Check sheet for the modelled part. Datum: model origin and axes. Units: mm. A direction names the side the tool comes from. Round coordinates to 2 decimals unless told otherwise and drop trailing zeros. Order: outer loops, then holes, each group sorted by start corner. A loop starts at its lowest first (then second) coordinate and runs counter-clockwise, first axis right, second up. Notation, with made-up numbers: (-24.5, -32.5) -> (-13.5, -32.5) arc R26 cw to (-13.5, -18.5) -> close; hole circle Ø11 at (36, -16). An arc over 180 degrees is marked (long way). Answer in a Markdown table with one row per item.
from build123d import *

# Parameters (mm, degrees)
SKETCH2_R           = 0.4
BOSS_EXTRUDE1_DEPTH = 0.5
SKETCH4_R           = 1
SKETCH4_R_2         = 0.5
CUT_EXTRUDE3_DEPTH  = 6


with BuildPart() as part:
    # Sketch1 → Revolve1 (revolve)
    with BuildSketch(Plane.XY, mode=Mode.PRIVATE) as revolve1_sk:
        Polygon((0, 0), (0, 1.5), (3, 1.5), (3, 1), (13, 1), (13, 0), align=None)
    revolve(revolve1_sk.sketch.rotate(Axis((0.124352332, 0, 0), (1, 0, 0)), 90), axis=Axis((0.124352332, 0, 0), (1, 0, 0)))

    # Sketch2 → Boss-Extrude1 (add, symmetric)
    with BuildSketch(Plane.XY):
        with BuildLine():
            Line((0, 0.75), (0, -0.75))
            Line((0, -0.75), (-3, -0.75))
            ThreePointArc((-3, -0.75), (-3.75, 0), (-3, 0.75))
            Line((-3, 0.75), (0, 0.75))
        make_face()
        with Locations((-3, 0)):
            Circle(SKETCH2_R, mode=Mode.SUBTRACT)
    extrude(amount=BOSS_EXTRUDE1_DEPTH, both=True)

    # Sketch4 → Cut-Extrude3 (cut)
    with BuildSketch(Plane(origin=(13, 0, 0), x_dir=(0, 0, -1), z_dir=(1, 0, 0))):
        with Locations(Location((0, 0, 0), (0, 0, 180))):
            Circle(SKETCH4_R)
        Circle(SKETCH4_R_2, mode=Mode.SUBTRACT)
    extrude(amount=-CUT_EXTRUDE3_DEPTH, mode=Mode.SUBTRACT)


solid = part.part
Item 1: Cross-section at A-A (y = 0). Record the boundary of the cut face in (x, z).
Result sheet:
| item | result |
|---|---|
| outline | (-3.75, -0.5) -> (-3.4, -0.5) -> (-3.4, 0.5) -> (-3.75, 0.5) -> close; (-2.6, -0.5) -> (0, -0.5) -> (0, -1.5) -> (3, -1.5) -> (3, -1) -> (7, -1) -> (7, -0.5) -> (13, -0.5) -> (13, 0.5) -> (7, 0.5) -> (7, 1) -> (3, 1) -> (3, 1.5) -> (0, 1.5) -> (0, 0.5) -> (-2.6, 0.5) -> close |
Item 2: Depth check by flat-ended pin: P1, Ø1.1, axis at x = -1, z = 0, coming from the -Y side; P2, Ø1, axis at y = 1, z = 1, coming from the -X side; P3, Ø0.8, axis at x = -1, z = 0, coming from the +Y side. Enter the tip coordinate at first touch or a pass-through.
Result sheet:
| item | result |
|---|---|
| P1 | stops at y = -0.75 |
| P2 | stops at x = 0 |
| P3 | stops at y = 0.75 |
Item 3: Cross-section at D-D (x = 8.5). Record the boundary of the cut face in (y, z).
Result sheet:
| item | result |
|---|---|
| outline | circle Ø1 at (0, 0) |
Item 4: Set-up check for faces 1 (the flat face through (-2, 0, -0.5)), 2 (the flat face through (-1, -0.75, 0)), 3 (the flat face through (-2, 0, 0.5)), 4 (the cylindrical face through (5, 1, 0)), 5 (the flat face through (-2, 0.75, 0)): record each of +Z, -Z, +X, -X, +Y, -Y from which the full face is reachable in a straight line by a thin tool's end or side.
Result sheet:
| item | result |
|---|---|
| face 1 | -Z, -X, +Y, -Y |
| face 2 | +Z, -Z, -X, -Y |
| face 3 | +Z, -X, +Y, -Y |
| face 4 | +X |
| face 5 | +Z, -Z, -X, +Y |
Item 5: Cross-section at C-C (z = 1.2). Record the boundary of the cut face in (x, y).
Result sheet:
| item | result |
|---|---|
| outline | (0, -0.9) -> (3, -0.9) -> (3, 0.9) -> (0, 0.9) -> close |
Item 6: Scan lines: line 1 (Y direction, x = -3, z = -0.2); line 2 (Y direction, x = 9.25, z = 0.05); line 3 (X direction, y = 0.1, z = -0.3). Record each from-to range of solid material in increasing order. Write a range as [from, to].
Result sheet:
| item | result |
|---|---|
| line 1 | y = [-0.75, -0.4], [0.4, 0.75] |
| line 2 | y = [-0.5, 0.5] |
| line 3 | x = [-3.74, -3.39], [-2.61, 13] |
Item 7: Cross-section at B-B (z = 0). Record the boundary of the cut face in (x, y).
Result sheet:
| item | result |
|---|---|
| outline | (-3, -0.75) -> (0, -0.75) -> (0, -1.5) -> (3, -1.5) -> (3, -1) -> (7, -1) -> (7, -0.5) -> (13, -0.5) -> (13, 0.5) -> (7, 0.5) -> (7, 1) -> (3, 1) -> (3, 1.5) -> (0, 1.5) -> (0, 0.75) -> (-3, 0.75) arc R0.75 ccw to start; hole circle Ø0.8 at (-3, 0) |
